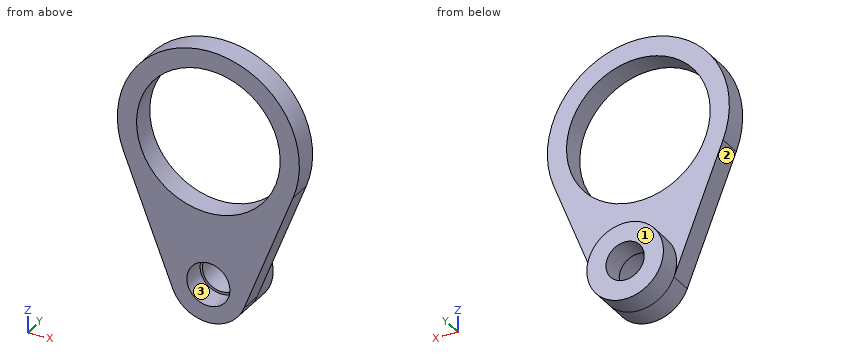
from build123d import *

# Parameters (mm, degrees)
BOSS_EXTRUDE1_DEPTH = 5
SKETCH2_R           = 8
BOSS_EXTRUDE2_DEPTH = 5
SKETCH3_R           = 4
SKETCH3_R_2         = 15
CUT_EXTRUDE1_DEPTH  = 39
SKETCH4_R           = 4.5
CUT_EXTRUDE2_DEPTH  = 5


with BuildPart() as part:
    # Sketch1 → Boss-Extrude1 (new body)
    with BuildSketch(Plane(origin=(0, 0, 0), x_dir=(1, 0, 0), z_dir=(0, 1, 0))):
        with BuildLine():
            Line((-7.44281906, 2.933333333), (-17.676695267, -23.033333333))
            ThreePointArc((-17.676695267, -23.033333333), (0, -49), (17.676695267, -23.033333333))
            Line((17.676695267, -23.033333333), (7.44281906, 2.933333333))
            ThreePointArc((7.44281906, 2.933333333), (0, 8), (-7.44281906, 2.933333333))
        make_face()
    extrude(amount=BOSS_EXTRUDE1_DEPTH)

    # Sketch2 → Boss-Extrude2 (add)
    with BuildSketch(Plane(origin=(0, 5, 0), x_dir=(1, 0, 0), z_dir=(0, 1, 0))):
        with Locations(Location((0, 0, 0), (0, 0, 158.489811733))):
            Circle(SKETCH2_R)
    extrude(amount=BOSS_EXTRUDE2_DEPTH)

    # Sketch3 → Cut-Extrude1 (cut)
    with BuildSketch(Plane(origin=(0, 10, 0), x_dir=(1, 0, 0), z_dir=(0, 1, 0))):
        with Locations(Location((0, 0, 0), (0, 0, 270))):
            Circle(SKETCH3_R)
        with Locations(Location((0, -30, 0), (0, 0, 270))):
            Circle(SKETCH3_R_2)
    extrude(amount=-CUT_EXTRUDE1_DEPTH, mode=Mode.SUBTRACT)

    # Sketch4 → Cut-Extrude2 (cut)
    with BuildSketch(Plane.XZ):
        with Locations(Location((0, 0, 0), (0, 0, 270))):
            Circle(SKETCH4_R)
    extrude(amount=-CUT_EXTRUDE2_DEPTH, mode=Mode.SUBTRACT)


solid = part.part
The model under review builds one solid part; all positions refer to its coordinate system, in mm. Face numbers are marked on the shaded views. Give positions to 0.01 mm unless a question says otherwise; leave off trailing zeros. Write each loop counter-clockwise with the first axis right and the second up, starting at its lowest first coordinate (ties: lowest second). Pieces come first, ordered by that corner, then holes.
1. Draft analysis for pull direction X (two halves, no side actions). For the marked faces 1, 2 and 3, state which applies: +X half, -X half, draft (parallel to the pull), parting line (faces both ways), or undercut.
2. Wall thickness on L1, parallel to X at y = 6.35, z = 0; L2, parallel to X at y = 2.8, z = 30; L3, parallel to Y at x = -7, z = 45: over which ranges is each line inside the solid? List them lowest first.
3. Add section C-C, the plane x = 0. Write out the cut boundary in (y, z), plus the area to 3 significant figures.
4. For P1, Ø2, axis at x = -2.5, y = 3.5, coming from the +Z side; P2, Ø1.5, axis at x = 14, y = 3, coming from the +Z side; P3, Ø2, axis at x = -8, z = 13.5, coming from the +Y side, all flat-tipped, find the tip position at first contact; note any pin that passes through.
5. Add section B-B, the plane x = -9. Write out the cut boundary in (y, z), plus the area to 3 significant figures.
6. Add section A-A, the plane z = 30. Write out the cut boundary in (x, y), plus the area to 3 significant figures.
7. Add section D-D, the plane y = 8. Write out the cut boundary in (x, z), plus the area to 3 significant figures.
Worked answers:
1. face 1: draft
1. face 2: -X half
1. face 3: undercut
2. L1: x = -8 to -4, 4 to 8
2. L2: x = -19 to -15, 15 to 19
2. L3: y = 0 to 5
3. outline: (0, -8) - (10, -8) - (10, -4) - (5, -4) - (5, -4.5) - (0, -4.5) - close; (0, 4.5) - (5, 4.5) - (5, 4) - (10, 4) - (10, 8) - (5, 8) - (5, 15) - (0, 15) - close; (0, 45) - (5, 45) - (5, 49) - (0, 49) - close
3. area: 130 mm2
4. P1: stops at z = 48.94
4. P2: stops at z = 43.62
4. P3: stops at y = 5
5. outline: (0, 1.02) - (5, 1.02) - (5, 18) - (0, 18) - close; (0, 42) - (5, 42) - (5, 46.73) - (0, 46.73) - close
5. area: 109 mm2
6. outline: (-19, 0) - (-15, 0) - (-15, 5) - (-19, 5) - close; (15, 0) - (19, 0) - (19, 5) - (15, 5) - close
6. area: 40.0 mm2
7. outline: circle Ø16 at (0, 0); hole circle Ø8 at (0, 0)
7. area: 151 mm2
